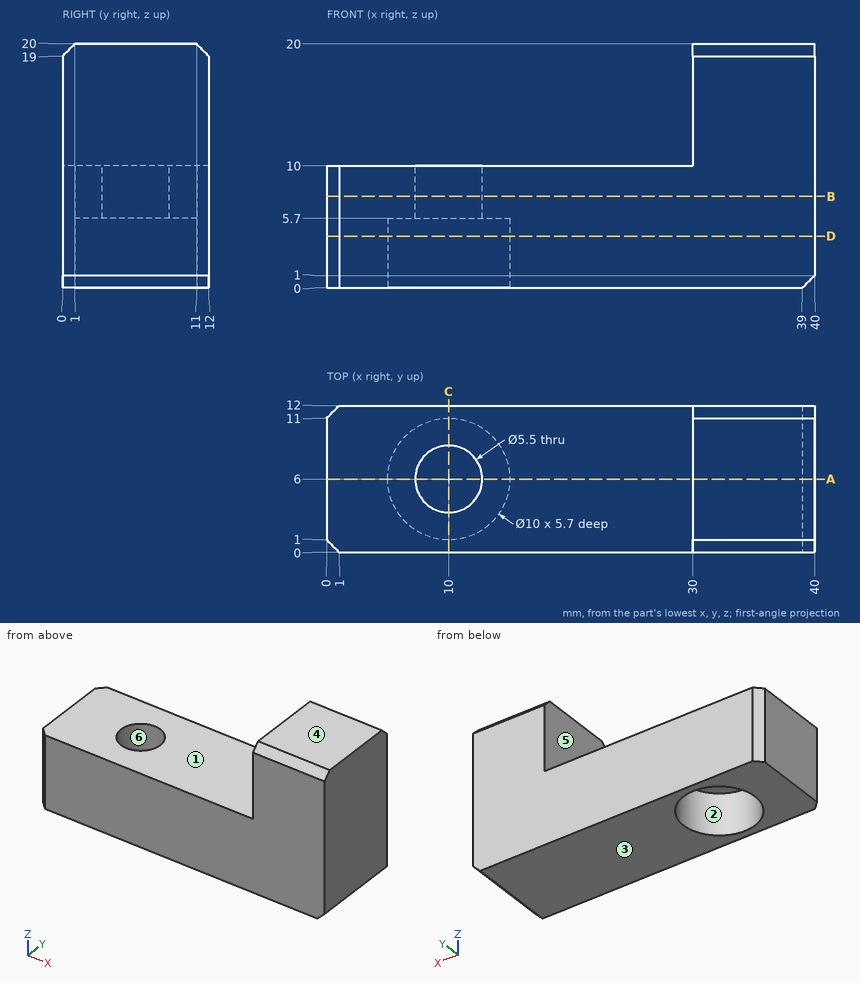
Design review of the part shown in the three views and the two pictorial views. Dimensions are in mm from the part's minimum x, y and z. A direction names the side the tool comes from. Round coordinates to 2 decimals unless told otherwise and drop trailing zeros. Write each loop counter-clockwise with the first axis right and the second up, starting at its lowest first coordinate (ties: lowest second). Pieces come first, ordered by that corner, then holes. Notation, with made-up numbers: M 70.5,32 L 110.5,32 A13 cw 110.5,41 Z; hole C 2.5,78.5 d8. An arc over 180 degrees is marked long. Use a Markdown table: item, result. Add a question column.
Q1. We need section B-B, the plane z = 7.5. State the section outline as (x, y) points.
Q2. The part is to be moulded in two halves that separate along X. For the marked faces 4, 5 and 6, say which applies: pulls with the +X half, pulls with the -X half, needs draft (parallel to the pull), parting line crosses it, or undercut.
Q3. Machinability: for the marked faces 1, 2 and 3, which of the approach directions +Z, -Z, +X, -X, +Y, -Y give a long, thin tool a straight path to every point of the face, cutting with its end or side? Answer none if there is none.
Q4. We need section A-A, the plane y = 6. State the section outline as (x, z) points, plus the area to 3 significant figures.
Q5. To check wall thickness, follow line 1 (X direction, y = 5.75, z = 19); line 2 (Z direction, x = 14.5, y = 7.75); line 3 (Y direction, x = 10, z = 6.8). State the ranges of each line that lie inside material, in increasing order.
Q6. We need section D-D, the plane z = 4.25. State the section outline as (x, y) points.
Q7. We need section C-C, the plane x = 10. State the section outline as (y, z) points, plus the area to 4 significant figures.
Q8. Insertion check: pin 1 (5 mm diameter, centred on y = 4, z = 14.5, fed in from -X); pin 2 (4 mm diameter, centred on x = 14.5, z = 12.5, fed in from -Y); pin 3 (6 mm diameter, centred on x = 10, y = 6, fed in from -Z). Each pin has a flat end and moves straight along its axis. Give the tip position at first contact, or say it passes through.
Findings below:
| question | item | result |
|---|---|---|
| 1 | outline | M 0,1 L 1,0 L 40,0 L 40,12 L 1,12 L 0,11 Z; hole C 10,6 d5.5 |
| 2 | face 4 | needs draft |
| 2 | face 5 | pulls with the -X half |
| 2 | face 6 | undercut |
| 3 | face 1 | +Z, -X, +Y, -Y |
| 3 | face 2 | -Z |
| 3 | face 3 | -Z, +X, -X, +Y, -Y |
| 4 | outline | M 0,0 L 5,0 L 5,5.7 L 7.25,5.7 L 7.25,10 L 0,10 Z; M 12.75,5.7 L 15,5.7 L 15,0 L 39,0 L 40,1 L 40,20 L 30,20 L 30,10 L 12.75,10 Z |
| 4 | area | 419 mm² |
| 5 | line 1 | x = 30 to 40 |
| 5 | line 2 | z = 5.7 to 10 |
| 5 | line 3 | y = 0 to 3.25, 8.75 to 12 |
| 6 | outline | M 0,1 L 1,0 L 40,0 L 40,12 L 1,12 L 0,11 Z; hole C 10,6 d10 |
| 7 | outline | M 0,0 L 1,0 L 1,5.7 L 3.25,5.7 L 3.25,10 L 0,10 Z; M 8.75,5.7 L 11,5.7 L 11,0 L 12,0 L 12,10 L 8.75,10 Z |
| 7 | area | 39.35 mm² |
| 8 | pin 1 | stops at x = 30 |
| 8 | pin 2 | passes through |
| 8 | pin 3 | stops at z = 5.7 |
